from build123d import *

# Parameters (mm, degrees)
SKETCH1_R           = 31.75
SKETCH1_R_2         = 2.667
BOSS_EXTRUDE1_DEPTH = 7.62
SKETCH2_R           = 6.604
SKETCH2_W           = 8.89
SKETCH2_H           = 17.78
CUT_EXTRUDE1_DEPTH  = 46.543269536
SKETCH3_R           = 2.667
CUT_EXTRUDE2_DEPTH  = 46.543269536
CIRPATTERN1_COUNT   = 4
SCALE1_SCALE        = 2


with BuildPart() as part:
    # Sketch1 → Boss-Extrude1 (new body)
    with BuildSketch(Plane(origin=(0, 0, 0), x_dir=(1, 0, 0), z_dir=(0, 1, 0))):
        with Locations(Location((0, 0, 0), (0, 0, 270))):
            Circle(SKETCH1_R)
        with Locations(Location((-15.24, 16.51, 0), (0, 0, 270))):
            Circle(SKETCH1_R_2, mode=Mode.SUBTRACT)
        with Locations(Location((15.24, 16.51, 0), (0, 0, 270))):
            Circle(SKETCH1_R_2, mode=Mode.SUBTRACT)
        with Locations(Location((15.24, -16.51, 0), (0, 0, 270))):
            Circle(SKETCH1_R_2, mode=Mode.SUBTRACT)
        with Locations(Location((-15.24, -16.51, 0), (0, 0, 270))):
            Circle(SKETCH1_R_2, mode=Mode.SUBTRACT)
    extrude(amount=-BOSS_EXTRUDE1_DEPTH)

    # Sketch2 → Cut-Extrude1 (cut, through all)
    with BuildSketch(Plane(origin=(0, 0, 0), x_dir=(1, 0, 0), z_dir=(0, 1, 0))):
        with Locations(Location((0, 0, 0), (0, 0, 270))):
            Circle(SKETCH2_R)
        with Locations((0, 31.75)):
            Rectangle(SKETCH2_W, SKETCH2_H)
    cut_extrude1 = extrude(amount=-CUT_EXTRUDE1_DEPTH, mode=Mode.SUBTRACT)

    # Sketch3 → Cut-Extrude2 (cut, through all)
    with BuildSketch(Plane(origin=(0, 0, 0), x_dir=(1, 0, 0), z_dir=(0, 1, 0))):
        with Locations(Location((-17.78, 0, 0), (0, 0, 270))):
            Circle(SKETCH3_R)
        with Locations(Location((0, 17.78, 0), (0, 0, 270))):
            Circle(SKETCH3_R)
        with Locations(Location((17.78, 0, 0), (0, 0, 270))):
            Circle(SKETCH3_R)
        with Locations(Location((0, -17.78, 0), (0, 0, 270))):
            Circle(SKETCH3_R)
    extrude(amount=-CUT_EXTRUDE2_DEPTH, mode=Mode.SUBTRACT)

    # CirPattern1: Cut-Extrude1 ×4 about axis
    cirpattern1_axis = Axis((0, 0, 0), (0, 1, 0))
    for i in range(1, CIRPATTERN1_COUNT):
        add(cut_extrude1.rotate(cirpattern1_axis, i * 360 / CIRPATTERN1_COUNT), mode=Mode.SUBTRACT)


with BuildPart() as part_1:
    # Scale1: scaled about (0, 0, 0)
    add(part.part.scale(SCALE1_SCALE))


solid = part_1.part
The model under review builds one solid part; all positions refer to its coordinate system, in mm. A direction names the side the tool comes from. Round coordinates to 2 decimals unless told otherwise and drop trailing zeros. Loops run counter-clockwise (first coordinate to the right, second up) from the corner with the lowest first, then second, coordinate; pieces in that order, holes last. Notation, with made-up numbers: (53.5, 35) -> (104.5, 35) arc R13 cw to (104.5, 43) -> close; hole circle Ø10 at (-31.75, -29.5). An arc over 180 degrees is marked (long way). One line per question, with ' | ' between items. Start each with the question number.
Item 1: For pin 1 (4.5 mm diameter, centred on y = -10, z = -52.5, fed in from -X); pin 2 (5 mm diameter, centred on y = -3.5, z = -3.5, fed in from +X); pin 3 (1 mm diameter, centred on x = -40.5, y = -2, fed in from -Z), all flat-tipped, find the tip position at first contact; note any pin that passes through.
Item 2: Add section C-C, the plane x = 0. Write out the cut boundary in (y, z), then the cut area to 3 significant figures.
Item 3: Add section D-D, the plane x = 42.5. Write out the cut boundary in (y, z).
Item 4: Add section B-B, the plane y = -11.5. Count the separate pieces of the cut face and the enclosed holes in it, then the cut area to 3 significant figures.
Item 5: Machinability: for faces 4 (the face through (8.89, -8, -54)), 5 (the face through (-54, -8, 8.89)), 6 (the face through (0, -8, 45.72)), 7 (the face through (45.72, -8, 0)), which of the approach directions +Z, -Z, +X, -X, +Y, -Y give a long, thin tool a straight path to every point of the face, cutting with its end or side? Answer none if there is none.
Item 6: Add section A-A, the plane z = 0. Write out the cut boundary in (x, y), then the cut area to 3 significant figures.
Item 7: Draft analysis for pull direction Z (two halves, no side actions). For faces 1 (the face through (-44.5, -7.5, -45.3)), 2 (the face through (54, -8, 8.89)), 3 (the face through (1, -15.24, -15)), state which applies: +Z half, -Z half, draft (parallel to the pull), parting line (faces both ways), or undercut.
Item 8: Wall thickness on line 1 along X through (y, z) = (-6.5, 0); line 2 along X through (y, z) = (-6, 35.56); line 3 along Z through (x, y) = (28, -7.75): over which ranges is each line inside the solid? List them lowest first. Write a range as [from, to].
Return value:
1) pin 1: stops at x = -38.82 | pin 2: stops at x = 45.72 | pin 3: stops at z = -49.32
2) outline: (-15.24, -45.72) -> (0, -45.72) -> (0, -40.89) -> (-15.24, -40.89) -> close; (-15.24, -30.23) -> (0, -30.23) -> (0, -13.21) -> (-15.24, -13.21) -> close; (-15.24, 13.21) -> (0, 13.21) -> (0, 30.23) -> (-15.24, 30.23) -> close; (-15.24, 40.89) -> (0, 40.89) -> (0, 45.72) -> (-15.24, 45.72) -> close | area: 666 mm2
3) outline: (-15.24, -47.18) -> (0, -47.18) -> (0, 47.18) -> (-15.24, 47.18) -> close
4) separate pieces: 1 | enclosed holes: 9 | area: 10,200 mm2
5) face 4: -Z, +Y, -Y | face 5: -X, +Y, -Y | face 6: +Z, +Y, -Y | face 7: +X, +Y, -Y
6) outline: (-45.72, -15.24) -> (-40.89, -15.24) -> (-40.89, 0) -> (-45.72, 0) -> close; (-30.23, -15.24) -> (-13.21, -15.24) -> (-13.21, 0) -> (-30.23, 0) -> close; (13.21, -15.24) -> (30.23, -15.24) -> (30.23, 0) -> (13.21, 0) -> close; (40.89, -15.24) -> (45.72, -15.24) -> (45.72, 0) -> (40.89, 0) -> close | area: 666 mm2
7) face 1: -Z half | face 2: undercut | face 3: draft
8) line 1: x = [-45.72, -40.89], [-30.23, -13.21], [13.21, 30.23], [40.89, 45.72] | line 2: x = [-52.61, -35.17], [-25.79, -5.33], [5.33, 25.79], [35.17, 52.61] | line 3: z = [-56.99, -37.74], [-28.3, 28.3], [37.74, 56.99]
